Check sheet for the drawn part. Datum: minimum x, y, z corner. Units: mm. Round coordinates to 2 decimals unless told otherwise and drop trailing zeros. Order: outer loops, then holes, each group sorted by start corner. A loop starts at its lowest first (then second) coordinate and runs counter-clockwise, first axis right, second up.
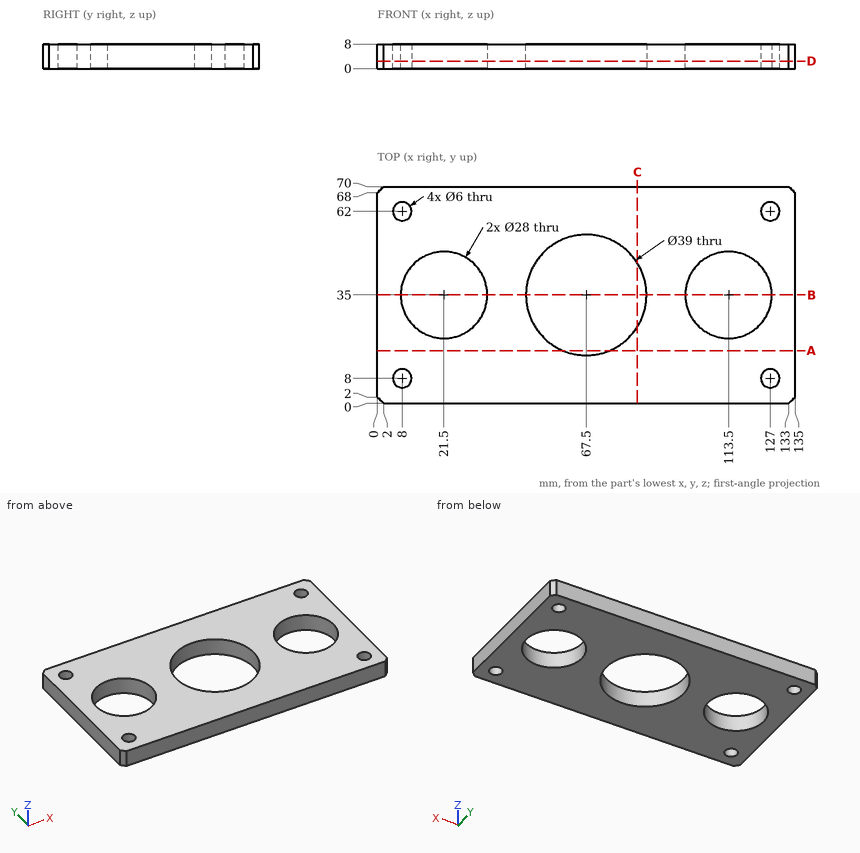
1) Sectioned sample at A-A on y = 17. Record the cut outline in (x, z).
2) Sectioned sample at C-C on x = 84. Record the cut outline in (y, z), and give its area (3 significant figures).
3) Sectioned sample at D-D on z = 2.5. Record the cut outline in (x, y), and give its area (3 significant figures).
4) Scan lines: line 1 (X direction, y = 44.5, z = 3.75); line 2 (X direction, y = 31, z = 3); line 3 (Y direction, x = 113.5, z = 5.75). Record each from-to range of solid material in increasing order.
5) Sectioned sample at B-B on y = 35. Record the cut outline in (x, z).
Values found:
1. outline: (0, 0) - (60, 0) - (60, 8) - (0, 8) - close; (75, 0) - (135, 0) - (135, 8) - (75, 8) - close
2. outline: (0, 0) - (24.61, 0) - (24.61, 8) - (0, 8) - close; (45.39, 0) - (70, 0) - (70, 8) - (45.39, 8) - close
2. area: 394 mm2
3. outline: (0, 2) - (2, 0) - (133, 0) - (135, 2) - (135, 68) - (133, 70) - (2, 70) - (0, 68) - close; hole circle Ø6 at (8, 8); hole circle Ø6 at (8, 62); hole circle Ø28 at (21.5, 35); hole circle Ø39 at (67.5, 35); hole circle Ø28 at (113.5, 35); hole circle Ø6 at (127, 8); hole circle Ø6 at (127, 62)
3. area: 6,900 mm2
4. line 1: x = 0 to 11.22, 31.78 to 50.47, 84.53 to 103.22, 123.78 to 135
4. line 2: x = 0 to 8.08, 34.92 to 48.41, 86.59 to 100.08, 126.92 to 135
4. line 3: y = 0 to 21, 49 to 70
5. outline: (0, 0) - (7.5, 0) - (7.5, 8) - (0, 8) - close; (35.5, 0) - (48, 0) - (48, 8) - (35.5, 8) - close; (87, 0) - (99.5, 0) - (99.5, 8) - (87, 8) - close; (127.5, 0) - (135, 0) - (135, 8) - (127.5, 8) - close
